Can you work these out from the model? Positions are in its coordinate system, mm. A direction names the side the tool comes from. Round coordinates to 2 decimals unless told otherwise and drop trailing zeros. Write each loop counter-clockwise with the first axis right and the second up, starting at its lowest first coordinate (ties: lowest second). Pieces come first, ordered by that corner, then holes. Notation, with made-up numbers: M -35.5,-18.5 L 9.5,-18.5 A26 cw 9.5,20.5 Z; hole C 10,76 d1. An arc over 180 degrees is marked long. Answer in a Markdown table with one row per item. Add a question column.
(1) For faces 5 (the face through (53, 95.5, 60)), 6 (the face through (102.18, -81.96, 12.04)), 7 (the face through (265, -85, 9)), which set-ups out of +Z, -Z, +X, -X, +Y, -Y let a thin tool reach every point of the face, with its end or its side?
(2) Suppose I cut it at D-D, the plane z = 75. Write out the boundary of the cut face in (x, y).
(3) If I drill on probe 1 along Y at (x, z) = (-169, 4); probe 2 along Y at (x, z) = (-99, 84); probe 3 along X at (y, z) = (16.5, 16.5), over which ranges is the centre line in solid material (lowest first)?
(4) Suppose I cut it at B-B, the plane x = 270.25. Write out the boundary of the cut face in (y, z).
(5) Suppose I cut it at A-A, the plane z = 99. Write out the boundary of the cut face in (x, y).
(6) I'm going to push flat-ended pins straight in: pin 1 (4.5 mm diameter, centred on x = 102, y = 88, fed in from -Z); pin 2 (10 mm diameter, centred on x = 89.5, y = 10.5, fed in from +Z); pin 3 (7 mm diameter, centred on x = 270.25, y = -85, fed in from -Z); pin 4 (19.5 mm diameter, centred on x = 105.5, y = -85, fed in from +Z). Where does each tip first touch, or does it pass through?
(7) If we mould it in two halves opening along X, with no side actions, what happens to faces 1 (the face through (-185, -1, 57)), 2 (the face through (-176.68, 82.13, 4.44)), 3 (the face through (285.5, -1, 57)), 4 (the face through (51, 97, 115))? For each: released by +X, released by -X, zero draft, split by the parting line, or undercut.
(8) Suppose I cut it at C-C, the plane x = 43. Write out the boundary of the cut face in (y, z), then the cut area to 3 significant figures.
from build123d import *

# Parameters (mm, degrees)
BOSS_EXTRUDE1_DEPTH                                  = 115
SHELL1_T                                             = -5
SKETCH5_R                                            = 5.5
CUT_EXTRUDE4_DEPTH                                   = 10
SKETCH6_R                                            = 2.05
CUT_EXTRUDE5_DEPTH                                   = 10
FILLET1_R                                            = 10
FILLET2_R                                            = 5
BOSS_EXTRUDE2_DEPTH                                  = 10
HOLE_SIZE_PER_SOCKET_HEAD_CAP_SCREW_TYPE_D           = 9
HOLE_SIZE_PER_SOCKET_HEAD_CAP_SCREW_TYPE_CBORE_D     = 15
HOLE_SIZE_PER_SOCKET_HEAD_CAP_SCREW_TYPE_CBORE_DEPTH = 9
SKETCH10_W                                           = 75
SKETCH10_H                                           = 191
CUT_EXTRUDE6_DEPTH                                   = 9
FILLET3_R                                            = 5


with BuildPart() as part:
    # Sketch1 → Boss-Extrude1 (new body)
    with BuildSketch(Plane.XY):
        Polygon((285.5, 0), (285.5, -100.5), (185, -100.5), (-185, -100.5), (-185, 100.5), (185, 100.5), (285.5, 100.5), align=None)
    extrude(amount=BOSS_EXTRUDE1_DEPTH)

    # Shell1
    shell1_openings = [part.faces().sort_by_distance(p)[0] for p in [
        (50.25, 0, 115),
    ]]
    offset(amount=SHELL1_T, openings=shell1_openings, kind=Kind.INTERSECTION)

    # Sketch5 → Cut-Extrude4 (cut)
    with BuildSketch(Plane(origin=(-84.5, 100.5, 0), x_dir=(0, 0, 1), z_dir=(0, 1, 0))):
        with Locations((75, 0)):
            Circle(SKETCH5_R)
    extrude(amount=-CUT_EXTRUDE4_DEPTH, mode=Mode.SUBTRACT)

    # Sketch6 → Cut-Extrude5 (cut)
    with BuildSketch(Plane.ZY.offset(185)):
        with Locations(Location((49, -37, 0), (0, 0, 270))):
            Circle(SKETCH6_R)
        with Locations(Location((49, 37, 0), (0, 0, 270))):
            Circle(SKETCH6_R)
        with Locations(Location((83, 37, 0), (0, 0, 270))):
            Circle(SKETCH6_R)
        with Locations(Location((83, -37, 0), (0, 0, 270))):
            Circle(SKETCH6_R)
    extrude(amount=-CUT_EXTRUDE5_DEPTH, mode=Mode.SUBTRACT)

    # Fillet1
    fillet1_edges = [part.edges().sort_by_distance(p)[0] for p in [
        (-185, -100.5, 57.5),
        (-185, 100.5, 57.5),
        (285.5, 100.5, 57.5),
        (285.5, -100.5, 57.5),
    ]]
    fillet(fillet1_edges, radius=FILLET1_R)

    # Fillet2
    fillet2_edges = [part.edges().sort_by_distance(p)[0] for p in [
        (280.5, -95.5, 60),
        (280.5, 95.5, 60),
        (-180, 95.5, 60),
        (-180, -95.5, 60),
    ]]
    fillet(fillet2_edges, radius=FILLET2_R)

    # Sketch7 → Boss-Extrude2 (add)
    with BuildSketch(Plane.XY.offset(5)):
        with BuildLine():
            Line((280.5, -90.5), (280.5, 90.5))
            ThreePointArc((280.5, 90.5), (279.035533906, 94.035533906), (275.5, 95.5))
            Line((275.5, 95.5), (-175, 95.5))
            ThreePointArc((-175, 95.5), (-178.535533906, 94.035533906), (-180, 90.5))
            Line((-180, 90.5), (-180, -90.5))
            ThreePointArc((-180, -90.5), (-178.535533906, -94.035533906), (-175, -95.5))
            Line((-175, -95.5), (275.5, -95.5))
            ThreePointArc((275.5, -95.5), (279.035533906, -94.035533906), (280.5, -90.5))
        make_face()
    extrude(amount=BOSS_EXTRUDE2_DEPTH)

    # Hole size per socket head cap screw type1 (through all)
    with Locations(Plane(origin=(0, 0, 0), x_dir=(-1, 0, 0), z_dir=(0, 0, -1))):
        with Locations((-270.25, -85), (-270.25, 85), (169.75, 85), (169.75, -85), (-105.5, -85), (-105.5, 85)):
            CounterBoreHole(HOLE_SIZE_PER_SOCKET_HEAD_CAP_SCREW_TYPE_D / 2, HOLE_SIZE_PER_SOCKET_HEAD_CAP_SCREW_TYPE_CBORE_D / 2, HOLE_SIZE_PER_SOCKET_HEAD_CAP_SCREW_TYPE_CBORE_DEPTH)

    # Sketch10 → Cut-Extrude6 (cut)
    with BuildSketch(Plane.XY.offset(15)):
        with Locations((57.5, 0)):
            Rectangle(SKETCH10_W, SKETCH10_H)
    extrude(amount=-CUT_EXTRUDE6_DEPTH, mode=Mode.SUBTRACT)

    # Fillet3
    fillet3_edges = [part.edges().sort_by_distance(p)[0] for p in [
        (20, -95.5, 10.5),
        (20, 95.5, 10.5),
        (95, 95.5, 10.5),
        (95, -95.5, 10.5),
    ]]
    fillet(fillet3_edges, radius=FILLET3_R)


solid = part.part
Calculated:
| question | item | result |
|---|---|---|
| 1 | face 5 | +Z |
| 1 | face 6 | +Z, -Z |
| 1 | face 7 | -Z |
| 2 | outline | M -185,-90.5 A10 ccw -175,-100.5 L 275.5,-100.5 A10 ccw 285.5,-90.5 L 285.5,90.5 A10 ccw 275.5,100.5 L -79,100.5 L -79,95.5 L 275.5,95.5 A5 cw 280.5,90.5 L 280.5,-90.5 A5 cw 275.5,-95.5 L -175,-95.5 A5 cw -180,-90.5 L -180,90.5 A5 cw -175,95.5 L -90,95.5 L -90,100.5 L -175,100.5 A10 ccw -185,90.5 Z |
| 3 | probe 1 | -100.5 to -92.46, -77.54 to 77.54, 92.46 to 100.5 |
| 3 | probe 2 | -100.5 to -95.5, 95.5 to 100.5 |
| 3 | probe 3 | -185 to -180, 280.5 to 285.5 |
| 4 | outline | M -100.5,0 L -92.5,0 L -92.5,9 L -89.5,9 L -89.5,15 L -95.5,15 L -95.5,115 L -100.5,115 Z; M -80.5,9 L -77.5,9 L -77.5,0 L 77.5,0 L 77.5,9 L 80.5,9 L 80.5,15 L -80.5,15 Z; M 89.5,9 L 92.5,9 L 92.5,0 L 100.5,0 L 100.5,115 L 95.5,115 L 95.5,15 L 89.5,15 Z |
| 5 | outline | M -185,-90.5 A10 ccw -175,-100.5 L 275.5,-100.5 A10 ccw 285.5,-90.5 L 285.5,90.5 A10 ccw 275.5,100.5 L -175,100.5 A10 ccw -185,90.5 Z; hole M -180,-90.5 A5 ccw -175,-95.5 L 275.5,-95.5 A5 ccw 280.5,-90.5 L 280.5,90.5 A5 ccw 275.5,95.5 L -175,95.5 A5 ccw -180,90.5 Z |
| 6 | pin 1 | z = 9 |
| 6 | pin 2 | z = 6 |
| 6 | pin 3 | through |
| 6 | pin 4 | z = 15 |
| 7 | face 1 | released by -X |
| 7 | face 2 | undercut |
| 7 | face 3 | released by +X |
| 7 | face 4 | zero draft |
| 8 | outline | M -100.5,0 L 100.5,0 L 100.5,115 L 95.5,115 L 95.5,6 L -95.5,6 L -95.5,115 L -100.5,115 Z |
| 8 | area | 2,300 mm² |
